from build123d import *

# Parameters (mm, degrees)
NUT_BODY_8MM_DEPTH     = 4
M12_TAPPED_HOLE1_D     = 12
EDGE_CHAMFER_1X45_SIZE = 1


with BuildPart() as part:
    # Slotted Nut Profile → Nut Body 8mm (new, symmetric)
    with BuildSketch(Plane.XY):
        with BuildLine():
            Line((-2, 12.338962679), (-2, 10.338962679))
            Line((-2, 10.338962679), (2, 10.338962679))
            Line((2, 10.338962679), (2, 12.338962679))
            ThreePointArc((2, 12.338962679), (8.838834765, 8.838834765), (12.338962679, 2))
            Line((12.338962679, 2), (10.338962679, 2))
            Line((10.338962679, 2), (10.338962679, -2))
            Line((10.338962679, -2), (12.338962679, -2))
            ThreePointArc((12.338962679, -2), (8.838834765, -8.838834765), (2, -12.338962679))
            Line((2, -12.338962679), (2, -10.338962679))
            Line((2, -10.338962679), (-2, -10.338962679))
            Line((-2, -10.338962679), (-2, -12.338962679))
            ThreePointArc((-2, -12.338962679), (-8.838834765, -8.838834765), (-12.338962679, -2))
            Line((-12.338962679, -2), (-10.338962679, -2))
            Line((-10.338962679, -2), (-10.338962679, 2))
            Line((-10.338962679, 2), (-12.338962679, 2))
            ThreePointArc((-12.338962679, 2), (-8.838834765, 8.838834765), (-2, 12.338962679))
        make_face()
    extrude(amount=NUT_BODY_8MM_DEPTH, both=True)

    # M12 Tapped Hole1 (through all)
    with Locations(Plane.XY.offset(4)):
        with Locations((0, 0)):
            Hole(M12_TAPPED_HOLE1_D / 2)

    # Edge Chamfer 1x45°
    edge_chamfer_1x45_edges = [part.edges().sort_by_distance(p)[0] for p in [
        (-8.838834765, 8.838834765, 4),
        (-8.838834765, -8.838834765, 4),
        (8.838834765, -8.838834765, 4),
        (8.838834765, 8.838834765, 4),
    ]]
    chamfer(edge_chamfer_1x45_edges, length=EDGE_CHAMFER_1X45_SIZE)


solid = part.part
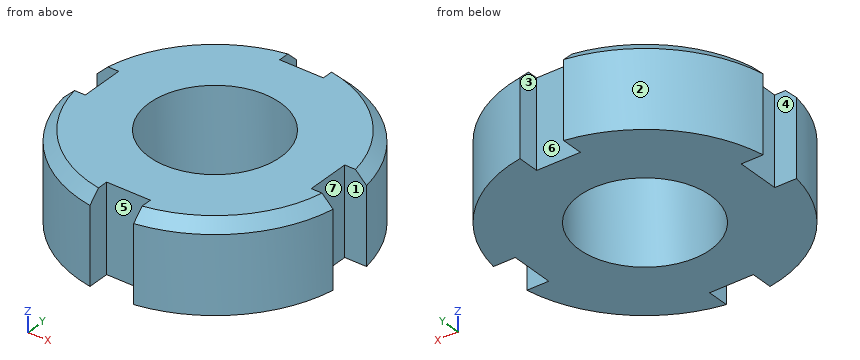
Here's how the part is built. I have some questions about the finished solid (model axes, mm). Face numbers are marked on the shaded views. A direction names the side the tool comes from. Give positions to 0.01 mm unless a question says otherwise; leave off trailing zeros. Write each loop counter-clockwise with the first axis right and the second up, starting at its lowest first coordinate (ties: lowest second). Pieces come first, ordered by that corner, then holes. Notation, with made-up numbers: (59.5, -30.5) -> (104.5, -30.5) arc R17 ccw to (104.5, -9.5) -> close; hole circle Ø10 at (-31, -33.5). An arc over 180 degrees is marked (long way). Use one line per item in the form item = value. Start each with the question number.
1. If I drill on L1, parallel to Y at x = 0, z = 1.75; L2, parallel to X at y = 0.5, z = 2.5; L3, parallel to X at y = 4.25, z = -2.5, over which ranges is the centre line in solid material (lowest first)?
2. Will these pins go through, and if not, where does the flat tip stop? pin 1 Ø1.6 at (x, z) = (11.5, 0.5) entering from +Y; pin 2 Ø1 at (x, z) = (-11.5, -0.5) entering from -Y; pin 3 Ø1.6 at (x, z) = (-11, 1.5) entering from +Y; pin 4 Ø9.5 at (x, y) = (0, 0) entering from +Z.
3. Imagine slicing it at C-C on z = 0. List the corners of the cut face in (x, y) for me.
4. Imagine slicing it at A-A on y = 0. List the corners of the cut face in (x, z) for me, plus the area to 3 significant figures.
5. On a 3-axis mill with a long thin cutter (end or side, diameter ignored), from which of +Z, -Z, +X, -X, +Y, -Y can I reach the whole of each face in a straight line? I mean the marked faces 4, 5, 6 and 7. Say none if no direction works.
6. Thinking about a two-plate mould opening in X: for the marked faces 1, 2 and 3, which applies, +X half, -X half, draft (parallel to the pull), parting line (faces both ways), or undercut?
Entries:
q1.L1 = -10.34 to -6, 6 to 10.34
q1.L2 = -10.34 to -5.98, 5.98 to 10.34
q1.L3 = -11.76 to -4.24, 4.24 to 11.76
q2.pin_1 = 6.46
q2.pin_2 = -5.94
q2.pin_3 = 7.23
q2.pin_4 = through
q3.outline = (-12.34, -2) arc R12.5 ccw to (-2, -12.34) -> (-2, -10.34) -> (2, -10.34) -> (2, -12.34) arc R12.5 ccw to (12.34, -2) -> (10.34, -2) -> (10.34, 2) -> (12.34, 2) arc R12.5 ccw to (2, 12.34) -> (2, 10.34) -> (-2, 10.34) -> (-2, 12.34) arc R12.5 ccw to (-12.34, 2) -> (-10.34, 2) -> (-10.34, -2) -> close; hole circle Ø12 at (0, 0)
q4.outline = (-10.34, -4) -> (-6, -4) -> (-6, 4) -> (-10.34, 4) -> close; (6, -4) -> (10.34, -4) -> (10.34, 4) -> (6, 4) -> close
q4.area = 69.4 mm²
q5.face_4 = +Z, -Z, -X
q5.face_5 = +Z, -Z, -Y
q5.face_6 = +Z, -Z, +Y
q5.face_7 = +Z, -Z, +X
q6.face_1 = draft
q6.face_2 = -X half
q6.face_3 = undercut
